For this review, take the finished solid that the model builds, in its own axes (mm). Round coordinates to 2 decimals unless told otherwise and drop trailing zeros. Loops run counter-clockwise (first coordinate to the right, second up) from the corner with the lowest first, then second, coordinate; pieces in that order, holes last. Notation, with made-up numbers: (57.25, 50.25) -> (75.25, 50.25) arc R15 cw to (75.25, 64.25) -> close; hole circle Ø2 at (-32, -0.75). An arc over 180 degrees is marked (long way). Use one line per item in the form item = value. Start each with the question number.
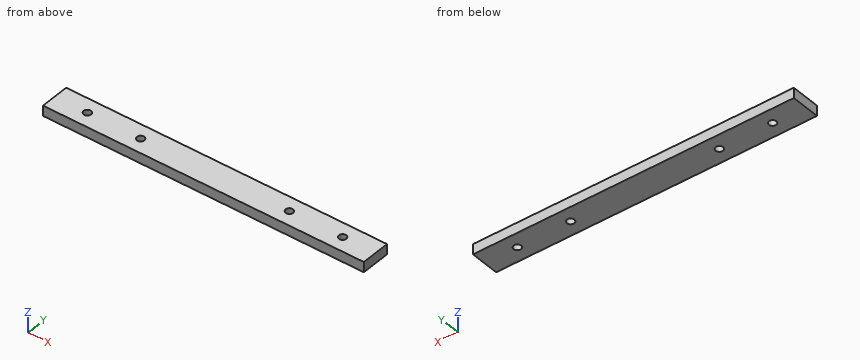
from build123d import *

# Parameters (mm, degrees)
SKETCH_1_W              = 440
SKETCH_1_H              = 40
EXTRUDE_1_DEPTH         = 14
HOLE_WIZARD_M12_1_D     = 10.2
HOLE_WIZARD_M12_1_DEPTH = 29.25
HOLE_WIZARD_M12_1_TIP   = 3.064389157


with BuildPart() as part:
    # 草图1 → 凸台-拉伸1 (new body)
    with BuildSketch(Plane.XY):
        with Locations((220, 20)):
            Rectangle(SKETCH_1_W, SKETCH_1_H)
    extrude(amount=EXTRUDE_1_DEPTH)

    # M12 螺纹孔1
    with Locations(Plane(origin=(45, 20, 14), x_dir=(1, 0, 0), z_dir=(0, 0, 1))):
        with Locations((0, 0), (73, 0), (350, 0), (277, 0)):
            Hole(HOLE_WIZARD_M12_1_D / 2, depth=HOLE_WIZARD_M12_1_DEPTH)
            with Locations((0, 0, -(HOLE_WIZARD_M12_1_DEPTH + HOLE_WIZARD_M12_1_TIP / 2))):  # 118° drill point
                Cone(0, HOLE_WIZARD_M12_1_D / 2, HOLE_WIZARD_M12_1_TIP, mode=Mode.SUBTRACT)


solid = part.part
Item 1: Take a section at C-C on x = 45. Give the boundary of the cut face in (y, z), plus the area to 3 significant figures.
Item 2: Take a section at B-B on y = 20. Give the boundary of the cut face in (x, z), plus the area to 3 significant figures.
Item 3: Wall thickness on line 1 (X direction, y = 19.5, z = 1); line 2 (Y direction, x = 118, z = 9); line 3 (X direction, y = 22, z = 3.25): over which ranges is each line inside the solid? List them lowest first.
Item 4: Take a section at A-A on z = 2.25. Give the boundary of the cut face in (x, y).
Results:
q1.outline = (0, 0) -> (14.9, 0) -> (14.9, 14) -> (0, 14) -> close; (25.1, 0) -> (40, 0) -> (40, 14) -> (25.1, 14) -> close
q1.area = 417 mm2
q2.outline = (0, 0) -> (39.9, 0) -> (39.9, 14) -> (0, 14) -> close; (50.1, 0) -> (112.9, 0) -> (112.9, 14) -> (50.1, 14) -> close; (123.1, 0) -> (316.9, 0) -> (316.9, 14) -> (123.1, 14) -> close; (327.1, 0) -> (389.9, 0) -> (389.9, 14) -> (327.1, 14) -> close; (400.1, 0) -> (440, 0) -> (440, 14) -> (400.1, 14) -> close
q2.area = 5,590 mm2
q3.line_1 = 0 to 39.92, 50.08 to 112.92, 123.08 to 316.92, 327.08 to 389.92, 400.08 to 440
q3.line_2 = 0 to 14.9, 25.1 to 40
q3.line_3 = 0 to 40.31, 49.69 to 113.31, 122.69 to 317.31, 326.69 to 390.31, 399.69 to 440
q4.outline = (0, 0) -> (440, 0) -> (440, 40) -> (0, 40) -> close; hole circle Ø10.2 at (45, 20); hole circle Ø10.2 at (118, 20); hole circle Ø10.2 at (322, 20); hole circle Ø10.2 at (395, 20)
